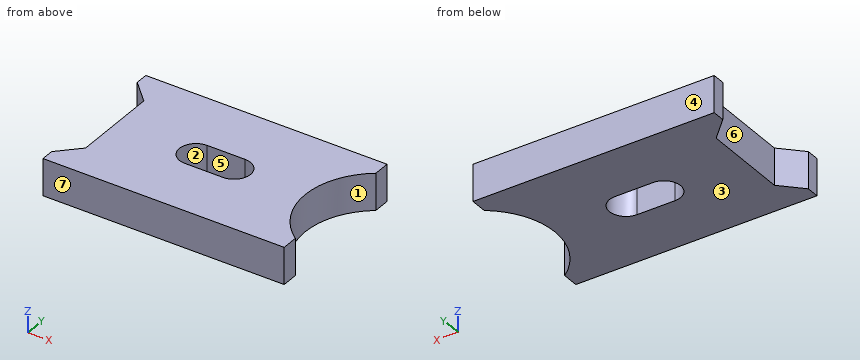
```python
from build123d import *

# Parameters (mm, degrees)
BOSS_EXTRUDE1_DEPTH = 14.5


with BuildPart() as part:
    # Sketch1 → Boss-Extrude1 (new body)
    with BuildSketch(Plane.XY):
        with BuildLine():
            ThreePointArc((47.5, 23.5), (35.5, 0), (47.5, -23.5))
            Line((47.5, -23.5), (47.5, -30))
            Line((47.5, -30), (-47.5, -30))
            Line((-47.5, -30), (-47.5, -25))
            Line((-47.5, -25), (-39.5, -17))
            Line((-39.5, -17), (-39.5, 17))
            Line((-39.5, 17), (-47.5, 25))
            Line((-47.5, 25), (-47.5, 30))
            Line((-47.5, 30), (47.5, 30))
            Line((47.5, 30), (47.5, 23.5))
        make_face()
        with BuildLine():
            Line((-7.5, -6.5), (7.5, -6.5))
            ThreePointArc((7.5, -6.5), (14, 0), (7.5, 6.5))
            Line((7.5, 6.5), (-7.5, 6.5))
            ThreePointArc((-7.5, 6.5), (-14, 0), (-7.5, -6.5))
        make_face(mode=Mode.SUBTRACT)
    extrude(amount=BOSS_EXTRUDE1_DEPTH)


solid = part.part
```
Source: CAD feature listing. Evaluate the final solid. Frame: model axes, mm. Face numbers are marked on the shaded views. A direction names the side the tool comes from. Coordinates: 2 decimals unless noted, no trailing zeros. Loops run counter-clockwise (first coordinate to the right, second up) from the corner with the lowest first, then second, coordinate; pieces in that order, holes last. Notation, with made-up numbers: M -10.5,-12 L 2.5,-12 A14 cw 2.5,2 Z; hole C 37.5,23 d10. An arc over 180 degrees is marked long. Use CSV: the item, a comma, the result in double quotes.
(1) Reachability of the marked faces 5, 6 and 7 from +Z, -Z, +X, -X, +Y, -Y: full face, straight path, thin tool, end or side. Return the list, or none.
Answers follow:
face 5,"+Z, -Z"
face 6,"+Z, -Z, -X"
face 7,"+Z, -Z, +X, -X, -Y"
(2) Cut plane A-A on x = -3.5. Return loops of the section in (y, z).
Answers follow:
outline,"M -30,0 L -6.5,0 L -6.5,14.5 L -30,14.5 Z; M 6.5,0 L 30,0 L 30,14.5 L 6.5,14.5 Z"
(3) Cut plane D-D on y = 18. Return loops of the section in (x, z), and give its area (3 significant figures).
Answers follow:
outline,"M -40.5,0 L 41.76,0 L 41.76,14.5 L -40.5,14.5 Z"
area,"1,190 mm²"
(4) Draft query along Y for the marked faces 1, 2, 3 and 4. Return one class per face: pulls with the +Y half, pulls with the -Y half, needs draft (parallel to the pull), parting line crosses it, or undercut.
Answers follow:
face 1,"undercut"
face 2,"undercut"
face 3,"needs draft"
face 4,"pulls with the +Y half"
(5) Cut plane B-B on y = 0. Return loops of the section in (x, z), and give its area (4 significant figures).
Answers follow:
outline,"M -39.5,0 L -14,0 L -14,14.5 L -39.5,14.5 Z; M 14,0 L 35.5,0 L 35.5,14.5 L 14,14.5 Z"
area,"681.5 mm²"
(6) Line query: line 1 (Y direction, x = -2.5, z = 6.25); line 2 (Y direction, x = -13, z = 2.75); line 3 (X direction, y = -22, z = 1.25). Output: solid intervals per line, ascending. Write a range as [from, to].
Answers follow:
line 1,"[-30, -6.5], [6.5, 30]"
line 2,"[-30, -3.46], [3.46, 30]"
line 3,"[-44.5, 45.6]"
(7) Cut plane C-C on z = 9.5. Return loops of the section in (x, y), and give its area (3 significant figures).
Answers follow:
outline,"M -47.5,-30 L 47.5,-30 L 47.5,-23.5 A29.01 cw 47.5,23.5 L 47.5,30 L -47.5,30 L -47.5,25 L -39.5,17 L -39.5,-17 L -47.5,-25 Z; hole M -7.5,-6.5 L 7.5,-6.5 A6.5 ccw 7.5,6.5 L -7.5,6.5 A6.5 ccw Z"
area,"4,640 mm²"
(8) Contact query for flat-ended pins moving along their axis: pin 1 (1.5 mm diameter, centred on y = 20, z = 9.5, fed in from +X); pin 2 (7 mm diameter, centred on y = 8, z = 5, fed in from -X); pin 3 (6 mm diameter, centred on y = 10.5, z = 12, fed in from +X). Output: stop coordinate, or through.
Answers follow:
pin 1,"x = 44.24"
pin 2,"x = -39.5"
pin 3,"x = 38.83"
